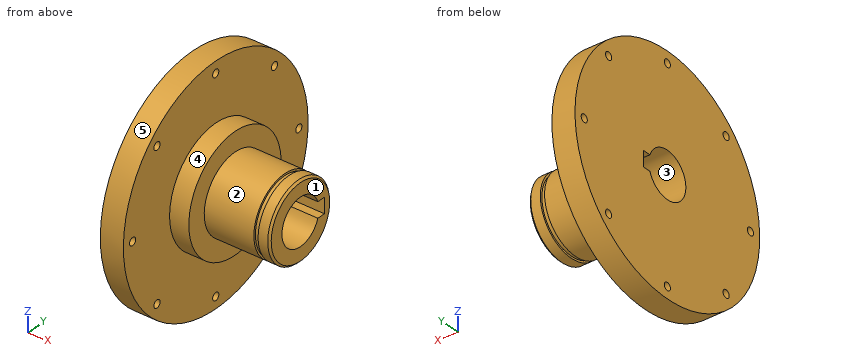
from build123d import *

# Parameters (mm, degrees)
SKETCH_1_W          = 12
SKETCH_1_H          = 60
SKETCH_2_W          = 10
SKETCH_2_H          = 30
SKETCH_3_W          = 34
SKETCH_3_H          = 20
CUT_EXTRUDE_2_DEPTH = 102.666120217
CUT_EXTRUDE_START   = 50
SKETCH_6_OUTSIDE_W  = 157.742
SKETCH_6_OUTSIDE_H  = 157.742
SKETCH_6_OUTSIDE_R  = 19
CUT_EXTRUDE_4_DEPTH = 2.2
SKETCH_7_R          = 2
CUT_EXTRUDE_5_DEPTH = 102.666120217
CHAMFER_2_SIZE      = 1


with BuildPart() as part:
    # 草图1 → 旋转-薄壁2 (revolve)
    with BuildSketch(Plane.XY, mode=Mode.PRIVATE) as revolve_2_sk:
        with Locations((6, 30)):
            Rectangle(SKETCH_1_W, SKETCH_1_H)
    revolve(revolve_2_sk.sketch.rotate(Axis((0, 0, 0), (1, 0, 0)), 90), axis=Axis((0, 0, 0), (1, 0, 0)))

    # 草图2 → 旋转-薄壁4 (revolve)
    with BuildSketch(Plane.XY, mode=Mode.PRIVATE) as revolve_4_sk:
        with Locations((17, 15)):
            Rectangle(SKETCH_2_W, SKETCH_2_H)
    revolve(revolve_4_sk.sketch.rotate(Axis((12, 0, 0), (1, 0, 0)), 90), axis=Axis((12, 0, 0), (1, 0, 0)))

    # 草图3 → 旋转-薄壁5 (revolve)
    with BuildSketch(Plane.XY, mode=Mode.PRIVATE) as revolve_5_sk:
        with Locations((39, 10)):
            Rectangle(SKETCH_3_W, SKETCH_3_H)
    revolve(revolve_5_sk.sketch.rotate(Axis((22, 0, 0), (1, 0, 0)), 90), axis=Axis((22, 0, 0), (1, 0, 0)))

    # 草图4 → 切除-拉伸2 (cut, through all)
    with BuildSketch(Plane(origin=(0, 0, 0), x_dir=(0, 0, -1), z_dir=(1, 0, 0))):
        with BuildLine():
            Line((-4, 15.6), (4, 15.6))
            Line((4, 15.6), (4, 11.313708499))
            ThreePointArc((4, 11.313708499), (0, -12), (-4, 11.313708499))
            Line((-4, 11.313708499), (-4, 15.6))
        make_face()
    extrude(amount=CUT_EXTRUDE_2_DEPTH, mode=Mode.SUBTRACT)

    # 草图6 outside → 切除-拉伸4 (cut)
    with BuildSketch(Plane(origin=(0, 0, 0), x_dir=(0, 0, -1), z_dir=(1, 0, 0)).offset(CUT_EXTRUDE_START)):
        Rectangle(SKETCH_6_OUTSIDE_W, SKETCH_6_OUTSIDE_H)
        Circle(SKETCH_6_OUTSIDE_R, mode=Mode.SUBTRACT)
    extrude(amount=-CUT_EXTRUDE_4_DEPTH, mode=Mode.SUBTRACT)

    # 草图7 → 切除-拉伸5 (cut, through all)
    with BuildSketch(Plane.ZY):
        with Locations((0, 54)):
            Circle(SKETCH_7_R)
        with Locations((38.183766184, 38.183766184)):
            Circle(SKETCH_7_R)
        with Locations((54, 0)):
            Circle(SKETCH_7_R)
        with Locations((38.183766184, -38.183766184)):
            Circle(SKETCH_7_R)
        with Locations((0, -54)):
            Circle(SKETCH_7_R)
        with Locations((-38.183766184, -38.183766184)):
            Circle(SKETCH_7_R)
        with Locations((-54, 0)):
            Circle(SKETCH_7_R)
        with Locations((-38.183766184, 38.183766184)):
            Circle(SKETCH_7_R)
    extrude(amount=-CUT_EXTRUDE_5_DEPTH, mode=Mode.SUBTRACT)

    # 倒角2
    chamfer_2_edges = [part.edges().sort_by_distance(p)[0] for p in [
        (56, 0, -20),
    ]]
    chamfer(chamfer_2_edges, length=CHAMFER_2_SIZE)


solid = part.part
Model file for the job. Use its own axes, mm. Face numbers are marked on the shaded views. A direction names the side the tool comes from. Coordinates: 2 decimals unless noted, no trailing zeros. Loops run counter-clockwise (first coordinate to the right, second up) from the corner with the lowest first, then second, coordinate; pieces in that order, holes last. Notation, with made-up numbers: (26, 54.5) -> (50, 54.5) arc R23 cw to (50, 92.5) -> close; hole circle Ø7 at (25.5, -40). An arc over 180 degrees is marked (long way). Use one line per item in the form item = value. Start each with the question number.
(1) Cut at A-A on y = 0. Give the number of separate pieces and of enclosed holes in the cut face, and give its area (3 significant figures).
(2) Tool access for the marked faces 4 and 5: list every direction of +Z, -Z, +X, -X, +Y, -Y with a clear straight run to the whole face (end or side of a thin tool).
(3) Pull direction Z, two halves, no side cores. Call the marked faces 1, 2 and 3: pulls with the +Z half, pulls with the -Z half, needs draft (parallel to the pull), parting line crosses it, or undercut.
(4) Cut at D-D on y = 54. Give the cut face in (x, z).
(5) Cut at C-C on x = 37. Give the cut face in (y, z), and give its area (3 significant figures).
(6) Probe probe 1 along Y at (x, z) = (6.25, 0); probe 2 along X at (y, z) = (43.5, 15.5); probe 3 along Y at (x, z) = (6, -3.5). List the from-to ranges inside material, lowest first. Write a range as from..to.
(7) Flat gauge pins, fed straight in: pin 1 (3.5 mm diameter, centred on y = 0, z = -54, fed in from +X); pin 2 (1 mm diameter, centred on x = 41.5, y = 12.5, fed in from -Z); pin 3 (12 mm diameter, centred on y = 44, z = 36.5, fed in from +X); pin 4 (3 mm diameter, centred on x = 29, z = 5, fed in from -Y). Where does each tip first touch, or does it go through?
Values:
q1.separate_pieces = 4
q1.enclosed_holes = 0
q1.area = 1,950 mm2
q2.face_4 = +X
q2.face_5 = +X, -X
q3.face_1 = needs draft
q3.face_2 = parting line crosses it
q3.face_3 = undercut
q4.outline = (0, -26.15) -> (12, -26.15) -> (12, -2) -> (0, -2) -> close; (0, 2) -> (12, 2) -> (12, 26.15) -> (0, 26.15) -> close
q5.outline = circle Ø40 at (0, 0); hole (11.31, -4) -> (15.6, -4) -> (15.6, 4) -> (11.31, 4) arc R12 ccw (long way) to start
q5.area = 774 mm2
q6.probe_1 = -60..-56, -52..-12, 15.6..52, 56..60
q6.probe_2 = 0..12
q6.probe_3 = -59.9..-11.48, 15.6..59.9
q7.pin_1 = through
q7.pin_2 = -16
q7.pin_3 = 12
q7.pin_4 = -19.69
